For this review, take the finished solid that the model builds, in its own axes (mm). Face numbers are marked on the shaded views. A direction names the side the tool comes from. Coordinates: 2 decimals unless noted, no trailing zeros. Loops run counter-clockwise (first coordinate to the right, second up) from the corner with the lowest first, then second, coordinate; pieces in that order, holes last.
1. Machinability: for the marked faces 1 and 2, which of the approach directions +Z, -Z, +X, -X, +Y, -Y give a long, thin tool a straight path to every point of the face, cutting with its end or side? Answer none if there is none.
2. Take a section at B-B, the plane z = 0. State the section outline as (x, y) points, then the cut area to 3 significant figures.
3. Take a section at D-D, the plane y = 51.5. State the section outline as (x, z) points, then the cut area to 3 significant figures.
4. Clearance check with flat-ended pins moving along their axes: P1, Ø10, axis at y = 34.5, z = -5.5, coming from the -X side; P2, Ø4, axis at x = -2, y = 9, coming from the -Z side. State where each tip first meets the part, or that it passes through.
5. Take a section at C-C, the plane y = 23. State the section outline as (x, z) points, then the cut area to 3 significant figures.
6. Take a section at A-A, the plane x = 0. State the section outline as (y, z) points, then the cut area to 3 significant figures.
7. Mouldability with a two-part tool opening along X and no side actions: class the marked faces 3, 4 and 5 as pulls with the +X half, pulls with the -X half, needs draft (parallel to the pull), parting line crosses it, or undercut.
8. To check wall thickness, follow probe 1 along Z at (x, y) = (0, 31.75); probe 2 along Z at (x, y) = (0, 17); probe 3 along X at (y, z) = (28, -1.75). State the ranges of each line that lie inside material, in increasing order.
```python
from build123d import *


with BuildPart() as part:
    # Pin Profile Sketch → Pin Body Revolve (revolve)
    with BuildSketch(Plane.XY, mode=Mode.PRIVATE) as pin_body_revolve_sk:
        with BuildLine():
            Line((5, 0), (5, 27))
            Line((5, 27), (4, 28))
            Line((4, 28), (4, 37))
            ThreePointArc((4, 37), (5.5, 38.5), (4, 40))
            Line((4, 40), (4, 47))
            ThreePointArc((4, 47), (5.5, 48.5), (4, 50))
            Line((4, 50), (4, 55))
            Line((4, 55), (6.989745962, 55))
            ThreePointArc((6.989745962, 55), (9.111066306, 54.121320344), (9.989745962, 52))
            Line((9.989745962, 52), (9.989745962, 20))
            Line((9.989745962, 20), (7.989745962, 20))
            Line((7.989745962, 20), (7.989745962, 5))
            Line((7.989745962, 5), (6.65, 0))
            Line((6.65, 0), (5, 0))
        make_face()
    revolve(pin_body_revolve_sk.sketch.rotate(Axis((0, 37.717557252, 0), (0, -1, 0)), 180), axis=Axis((0, 37.717557252, 0), (0, -1, 0)))


solid = part.part
```
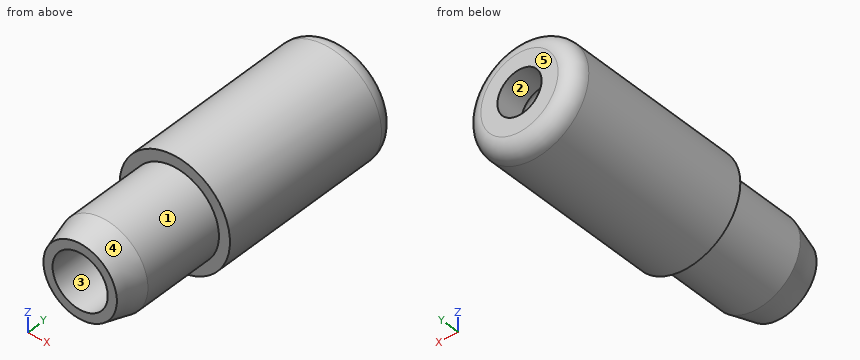
Results list:
1. face 1: -Y
1. face 2: +Y, -Y
2. outline: (-9.99, 20) - (-7.99, 20) - (-7.99, 5) - (-6.65, 0) - (-5, 0) - (-5, 27) - (-4, 28) - (-4, 37) arc R1.5 cw to (-4, 40) - (-4, 47) arc R1.5 cw to (-4, 50) - (-4, 55) - (-6.99, 55) arc R3 ccw to (-9.99, 52) - close; (4, 28) - (5, 27) - (5, 0) - (6.65, 0) - (7.99, 5) - (7.99, 20) - (9.99, 20) - (9.99, 52) arc R3 ccw to (6.99, 55) - (4, 55) - (4, 50) arc R1.5 cw to (4, 47) - (4, 40) arc R1.5 cw to (4, 37) - close
2. area: 499 mm2
3. outline: circle Ø19.98 at (0, 0); hole circle Ø8 at (0, 0)
3. area: 263 mm2
4. P1: stops at x = -9.98
4. P2: stops at z = -7.99
5. outline: circle Ø19.98 at (0, 0); hole circle Ø10 at (0, 0)
5. area: 235 mm2
6. outline: (0, -6.65) - (5, -7.99) - (20, -7.99) - (20, -9.99) - (52, -9.99) arc R3 ccw to (55, -6.99) - (55, -4) - (50, -4) arc R1.5 cw to (47, -4) - (40, -4) arc R1.5 cw to (37, -4) - (28, -4) - (27, -5) - (0, -5) - close; (0, 5) - (27, 5) - (28, 4) - (37, 4) arc R1.5 cw to (40, 4) - (47, 4) arc R1.5 cw to (50, 4) - (55, 4) - (55, 6.99) arc R3 ccw to (52, 9.99) - (20, 9.99) - (20, 7.99) - (5, 7.99) - (0, 6.65) - close
6. area: 499 mm2
7. face 3: undercut
7. face 4: parting line crosses it
7. face 5: needs draft
8. probe 1: z = -9.99 to -4, 4 to 9.99
8. probe 2: z = -7.99 to -5, 5 to 7.99
8. probe 3: x = -9.84 to -3.6, 3.6 to 9.84
